Could you check a few things on this model? Use its own coordinates, in mm. Face numbers are marked on the shaded views. A direction names the side the tool comes from. Round coordinates to 2 decimals unless told otherwise and drop trailing zeros. Order: outer loops, then holes, each group sorted by start corner. A loop starts at its lowest first (then second) coordinate and runs counter-clockwise, first axis right, second up.
```python
from build123d import *

# Parameters (mm, degrees)
SKETCH1_W           = 100
SKETCH1_H           = 100
BOSS_EXTRUDE1_DEPTH = 5
SKETCH2_R           = 10
BOSS_EXTRUDE2_DEPTH = 25
SKETCH3_W           = 50
SKETCH3_H           = 30
CUT_EXTRUDE1_DEPTH  = 130
SKETCH4_R           = 25
BOSS_EXTRUDE3_DEPTH = 400
CUT_EXTRUDE2_START  = -70
CUT_EXTRUDE2_DEPTH  = 70
SKETCH7_W           = 140
SKETCH7_H           = 70
BOSS_EXTRUDE4_DEPTH = 10


with BuildPart() as part:
    # Sketch1 → Boss-Extrude1 (new, symmetric)
    with BuildSketch(Plane.XY):
        Rectangle(SKETCH1_W, SKETCH1_H)
    extrude(amount=BOSS_EXTRUDE1_DEPTH, both=True)

    # Sketch2 → Boss-Extrude2 (add, symmetric)
    with BuildSketch(Plane(origin=(0, 0, 0), x_dir=(1, 0, 0), z_dir=(0, 1, 0))):
        with BuildLine():
            Line((-25, 5), (25, 5))
            Line((25, 5), (25, 65))
            ThreePointArc((25, 65), (0, 90), (-25, 65))
            Line((-25, 65), (-25, 5))
        make_face()
        with Locations(Location((0, 65, 0), (0, 0, 270))):
            Circle(SKETCH2_R, mode=Mode.SUBTRACT)
    extrude(amount=BOSS_EXTRUDE2_DEPTH, both=True)

    # Sketch3 → Cut-Extrude1 (cut)
    with BuildSketch(Plane(origin=(0, 0, -5), x_dir=(-1, 0, 0), z_dir=(0, 0, -1))):
        Rectangle(SKETCH3_W, SKETCH3_H)
    extrude(amount=CUT_EXTRUDE1_DEPTH, mode=Mode.SUBTRACT)

    # Sketch4 → Boss-Extrude3 (add)
    with BuildSketch(Plane.XY.offset(5)):
        with Locations(Location((0, 0, 0), (0, 0, 180))):
            Circle(SKETCH4_R)
    extrude(amount=BOSS_EXTRUDE3_DEPTH)

    # Sketch5 → Cut-Extrude2 (cut)
    with BuildSketch(Plane.XY.offset(405).offset(CUT_EXTRUDE2_START)):
        with BuildLine():
            Line((0, 25), (0, -25))
            ThreePointArc((0, -25), (25, 0), (0, 25))
        make_face()
    extrude(amount=CUT_EXTRUDE2_DEPTH, mode=Mode.SUBTRACT)

    # Sketch7 → Boss-Extrude4 (add)
    with BuildSketch(Plane(origin=(0, 0, 0), x_dir=(0, 0, -1), z_dir=(1, 0, 0))):
        with Locations((-405, 0)):
            Rectangle(SKETCH7_W, SKETCH7_H)
    extrude(amount=BOSS_EXTRUDE4_DEPTH)


solid = part.part
```
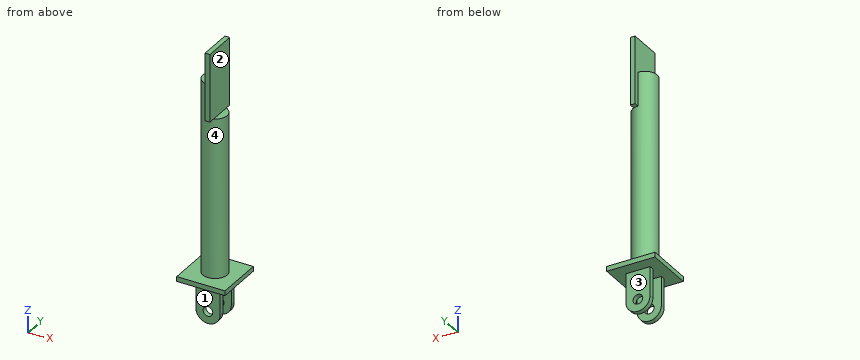
Q1. For the marked faces 1, 2, 3 and 4, which set-ups out of +Z, -Z, +X, -X, +Y, -Y let a thin tool reach every point of the face, with its end or its side?
Q2. Imagine slicing it at B-B, the plane x = -15. Please give me the cut outline in (y, z), then the cut area to 3 significant figures.
Q3. For P1, Ø25, axis at x = -2, z = -35.5, coming from the -Y side; P2, Ø15, axis at x = 10.5, z = -67.5, coming from the +Y side; P3, Ø12, axis at y = 23.5, z = 82, coming from the +X side, each with a flat end and sliding along its axis, tell me the tip position at first contact or that it passes through.
Q4. Imagine slicing it at A-A, the plane y = 0. Please give me the cut outline in (x, z), then the cut area to 4 significant figures.
Q5. Imagine slicing it at D-D, the plane z = 319. Please give me the cut outline in (x, y), then the cut area to 3 significant figures.
Q6. Imagine slicing it at C-C, the plane z = 441. Please give me the cut outline in (x, y).
Q7. I need wall thicknesses on L1, parallel to X at y = -18, z = -65; L2, parallel to Z at x = 46.5, y = -24.5; L3, parallel to Z at x = 2.5, y = 23. Which ranges of each line are inside material? Lowest first, please.
Filled in:
1. face 1: -Z, +X, -X, -Y
1. face 2: +Z, +X, +Y, -Y
1. face 3: -Z, +X, -X, +Y
1. face 4: none
2. outline: (-50, -5) - (-25, -5) - (-25, -85) - (-15, -85) - (-15, -5) - (15, -5) - (15, -85) - (25, -85) - (25, -5) - (50, -5) - (50, 5) - (20, 5) - (20, 405) - (-20, 405) - (-20, 5) - (-50, 5) - close
2. area: 18,600 mm2
3. P1: stops at y = -25
3. P2: stops at y = 25
3. P3: stops at x = 17.85
4. outline: (-50, -5) - (50, -5) - (50, 5) - (25, 5) - (25, 335) - (10, 335) - (10, 475) - (0, 475) - (0, 405) - (-25, 405) - (-25, 5) - (-50, 5) - close
4. area: 20,650 mm2
5. outline: circle Ø50 at (0, 0)
5. area: 1,960 mm2
6. outline: (0, -35) - (10, -35) - (10, 35) - (0, 35) - close
7. L1: x = -25 to -10, 10 to 25
7. L2: z = -5 to 5
7. L3: z = -89.87 to -74.68, -55.32 to 475
